from build123d import *

# Parameters (mm, degrees)
SKETCH1_W           = 40
SKETCH1_H           = 40
SKETCH1_W_2         = 36
SKETCH1_H_2         = 36
BOSS_EXTRUDE1_DEPTH = 95
FILLET1_R           = 2
FILLET2_R           = 4


with BuildPart() as part:
    # Sketch1 → Boss-Extrude1 (new body)
    with BuildSketch(Plane.XY):
        Rectangle(SKETCH1_W, SKETCH1_H)
        Rectangle(SKETCH1_W_2, SKETCH1_H_2, mode=Mode.SUBTRACT)
    extrude(amount=BOSS_EXTRUDE1_DEPTH)

    # Fillet1
    fillet1_edges = [part.edges().sort_by_distance(p)[0] for p in [
        (18, -18, 47.5),
        (18, 18, 47.5),
        (-18, 18, 47.5),
        (-18, -18, 47.5),
    ]]
    fillet(fillet1_edges, radius=FILLET1_R)

    # Fillet2
    fillet2_edges = [part.edges().sort_by_distance(p)[0] for p in [
        (20, -20, 47.5),
        (-20, -20, 47.5),
        (-20, 20, 47.5),
        (20, 20, 47.5),
    ]]
    fillet(fillet2_edges, radius=FILLET2_R)


solid = part.part
Design review of the part built by this model. Coordinates are the model's own, in mm. A direction names the side the tool comes from. Give positions to 0.01 mm unless a question says otherwise; leave off trailing zeros. Write each loop counter-clockwise with the first axis right and the second up, starting at its lowest first coordinate (ties: lowest second). Pieces come first, ordered by that corner, then holes. Notation, with made-up numbers: M 78.5,49.25 L 92.5,49.25 A23 ccw 92.5,77.25 Z; hole C 70,-22.5 d9. An arc over 180 degrees is marked long. Return JSON: item names as keys, results as strings. Group by question number.
Item 1: Take a section at A-A (x = -2). Give the boundary of the cut face in (y, z), plus the area to 3 significant figures.
Item 2: Tool access review of faces 1 (the cylindrical face through (-18.859, 18.797, 48.165)), 2 (the cylindrical face through (-17.4, -17.43, 48.16)): name each direction out of +Z, -Z, +X, -X, +Y, -Y from which nothing blocks a thin tool from reaching the whole face with its end or side.
Item 3: The part is to be moulded in two halves that separate along Y. For faces 3 (the cylindrical face through (18.797, -18.859, 48.165)), 4 (the flat face through (0, 20, 47)), 5 (the cylindrical face through (17.43, 17.4, 48.16)), 6 (the flat face through (0, -18, 47)), say which applies: pulls with the +Y half, pulls with the -Y half, needs draft (parallel to the pull), parting line crosses it, or undercut.
Item 4: Wall thickness on line 1 along Y through (x, z) = (10, 36); line 2 along Y through (x, z) = (16.5, 48.5): over which ranges is each line inside the solid? List them lowest first.
Item 5: Take a section at C-C (z = 10.5). Give the boundary of the cut face in (x, y), plus the area to 3 significant figures.
Return value:
{
 "1": {"outline": "M -20,0 L -18,0 L -18,95 L -20,95 Z; M 18,0 L 20,0 L 20,95 L 18,95 Z", "area": "380 mm2"},
 "2": {"face 1": "+Z, -Z, -X, +Y", "face 2": "+Z, -Z"},
 "3": {"face 3": "pulls with the -Y half", "face 4": "pulls with the +Y half", "face 5": "undercut", "face 6": "undercut"},
 "4": {"line 1": "y = -20 to -18, 18 to 20", "line 2": "y = -19.97 to -17.94, 17.94 to 19.97"},
 "5": {"outline": "M -20,-16 A4 ccw -16,-20 L 16,-20 A4 ccw 20,-16 L 20,16 A4 ccw 16,20 L -16,20 A4 ccw -20,16 Z; hole M -18,-16 A2 ccw -16,-18 L 16,-18 A2 ccw 18,-16 L 18,16 A2 ccw 16,18 L -16,18 A2 ccw -18,16 Z", "area": "294 mm2"}
}
